```python
from build123d import *

# Parameters (mm, degrees)
EXTRUDE_1_DEPTH     = 40
CUT_EXTRUDE_1_DEPTH = 40
SKETCH_3_W          = 5
SKETCH_3_H          = 40
EXTRUDE_3_DEPTH     = 6


with BuildPart() as part:
    # 草图1 → 凸台-拉伸1 (new body)
    with BuildSketch(Plane.XY):
        with BuildLine():
            Line((0, 0), (5, 0))
            Line((5, 0), (5, 261))
            ThreePointArc((5, 261), (3.70593121, 267.892024376), (0, 273.845232579))
            Line((0, 273.845232579), (-3.684210526, 270.464908216))
            ThreePointArc((-3.684210526, 270.464908216), (-0.953524372, 266.078333751), (0, 261))
            Line((0, 261), (0, 0))
        make_face()
    extrude(amount=EXTRUDE_1_DEPTH)

    # 草图2 → 切除-拉伸1 (cut)
    with BuildSketch(Plane(origin=(5, 0, 0), x_dir=(0, 0, -1), z_dir=(1, 0, 0))):
        Polygon((-20, 273.845232579), (-25, 273.845232579), (-25, 243.845232579), (-15, 243.845232579), (-15, 273.845232579), align=None)
    extrude(amount=-CUT_EXTRUDE_1_DEPTH, mode=Mode.SUBTRACT)

    # 草图3 → 凸台-拉伸3 (add)
    with BuildSketch(Plane.XZ):
        with Locations((2.5, 20)):
            Rectangle(SKETCH_3_W, SKETCH_3_H)
    extrude(amount=EXTRUDE_3_DEPTH)


solid = part.part
```
Here's how the part is built. I have some questions about the finished solid (model axes, mm). A direction names the side the tool comes from. Coordinates: 2 decimals unless noted, no trailing zeros. Order: outer loops, then holes, each group sorted by start corner. A loop starts at its lowest first (then second) coordinate and runs counter-clockwise, first axis right, second up. Notation, with made-up numbers: (-11, 1.25) -> (17, 1.25) arc R22 ccw to (17, 39.25) -> close; hole circle Ø7 at (65.5, -5). An arc over 180 degrees is marked (long way). Return JSON: item names as keys, results as strings.
1) If we section it at D-D on y = 87.5: List the corners of the cut face in (x, z) for me, plus the area to 3 significant figures.
Conclusion:
{"outline": "(0, 0) -> (5, 0) -> (5, 40) -> (0, 40) -> close", "area": "200 mm²"}
2) Thinking about a two-plate mould opening in Z: for faces 3 (the flat face through (2, 259, 15)), 4 (the flat face through (0, 129, 20)), 5 (the flat face through (3, 136, 40)), which applies, +Z half, -Z half, draft (parallel to the pull), parting line (faces both ways), or undercut?
Conclusion:
{"face 3": "undercut", "face 4": "draft", "face 5": "+Z half"}
3) On a 3-axis mill with a long thin cutter (end or side, diameter ignored), from which of +Z, -Z, +X, -X, +Y, -Y can I reach the whole of each face in a straight line? I mean faces 1 (the flat face through (2, 259, 25)), 2 (the cylindrical face through (3.74, 267.8, 32.39)). Say none if no direction works.
Conclusion:
{"face 1": "+X, -X, +Y", "face 2": "+Z, -Z, +X, +Y"}
4) If I drill on probe 1 along X at (y, z) = (30, 11); probe 2 along Y at (x, z) = (2.5, 6); probe 3 along Y at (x, z) = (2.5, 23), over which ranges is the centre line in solid material (lowest first)?
Conclusion:
{"probe 1": "x = 0 to 5", "probe 2": "y = -6 to 270.42", "probe 3": "y = -6 to 243.85"}
5) If we section it at A-A on y = 251: List the corners of the cut face in (x, z) for me, plus the area to 3 significant figures.
Conclusion:
{"outline": "(0, 0) -> (5, 0) -> (5, 15) -> (0, 15) -> close; (0, 25) -> (5, 25) -> (5, 40) -> (0, 40) -> close", "area": "150 mm²"}
6) If we section it at B-B on z = 34.5: List the corners of the cut face in (x, y) for me, plus the area to 3 significant figures.
Conclusion:
{"outline": "(-3.68, 270.46) arc R14 cw to (0, 261) -> (0, -6) -> (5, -6) -> (5, 261) arc R19 ccw to (0, 273.85) -> close", "area": "1,400 mm²"}
7) If we section it at C-C on x = -2: List the corners of the cut face in (y, z) for me.
Conclusion:
{"outline": "(268.21, 0) -> (272.01, 0) -> (272.01, 15) -> (268.21, 15) -> close; (268.21, 25) -> (272.01, 25) -> (272.01, 40) -> (268.21, 40) -> close"}
8) I'm going to push flat-ended pins straight in: P1, Ø1.5, axis at x = 2.5, z = 20, coming from the +Y side; P2, Ø3, axis at x = 1, y = 167, coming from the -Z side; P3, Ø6, axis at y = 214, z = 9.5, coming from the -X side. Where does each tip first touch, or does it pass through?
Conclusion:
{"P1": "stops at y = 243.85", "P2": "stops at z = 0", "P3": "stops at x = 0"}
